Source: CAD feature listing. Evaluate the final solid. Frame: model axes, mm. Face numbers are marked on the shaded views. Give positions to 0.01 mm unless a question says otherwise; leave off trailing zeros. Loops run counter-clockwise (first coordinate to the right, second up) from the corner with the lowest first, then second, coordinate; pieces in that order, holes last. Notation, with made-up numbers: M 24,-25 L 73,-25 A20 cw 73,-13 Z; hole C 84.5,10 d2. An arc over 180 degrees is marked long. Put each result on its own line as item: value.
from build123d import *

# Parameters (mm, degrees)
SKETCH1_R           = 95
SKETCH1_R_2         = 67.5
BOSS_EXTRUDE1_DEPTH = 25
CUT_EXTRUDE1_START  = -10
SKETCH2_R           = 95
SKETCH2_R_2         = 90
CUT_EXTRUDE1_DEPTH  = 10
SKETCH3_R           = 5.75
CUT_EXTRUDE2_DEPTH  = 17.5
CHAMFER1_SIZE       = 2


with BuildPart() as part:
    # Sketch1 → Boss-Extrude1 (new body)
    with BuildSketch(Plane(origin=(0, 0, 0), x_dir=(0, 0, -1), z_dir=(1, 0, 0))):
        Circle(SKETCH1_R)
        Circle(SKETCH1_R_2, mode=Mode.SUBTRACT)
    extrude(amount=BOSS_EXTRUDE1_DEPTH)

    # Sketch2 → Cut-Extrude1 (cut)
    with BuildSketch(Plane(origin=(25, 0, 0), x_dir=(0, 0, -1), z_dir=(1, 0, 0)).offset(CUT_EXTRUDE1_START)):
        Circle(SKETCH2_R)
        Circle(SKETCH2_R_2, mode=Mode.SUBTRACT)
    extrude(amount=CUT_EXTRUDE1_DEPTH, mode=Mode.SUBTRACT)

    # Sketch3 → Cut-Extrude2 (cut)
    with BuildSketch(Plane.ZY):
        with Locations((40.25, -69.715045005)):
            Circle(SKETCH3_R)
        with Locations((80.5, 0)):
            Circle(SKETCH3_R)
        with Locations((-40.25, -69.715045005)):
            Circle(SKETCH3_R)
        with Locations((-80.5, 0)):
            Circle(SKETCH3_R)
        with Locations((-40.25, 69.715045005)):
            Circle(SKETCH3_R)
        with Locations((40.25, 69.715045005)):
            Circle(SKETCH3_R)
    extrude(amount=-CUT_EXTRUDE2_DEPTH, mode=Mode.SUBTRACT)

    # Chamfer1
    chamfer1_edges = [part.edges().sort_by_distance(p)[0] for p in [
        (25, 0, 90),
        (0, 0, 67.5),
    ]]
    chamfer(chamfer1_edges, length=CHAMFER1_SIZE)


solid = part.part
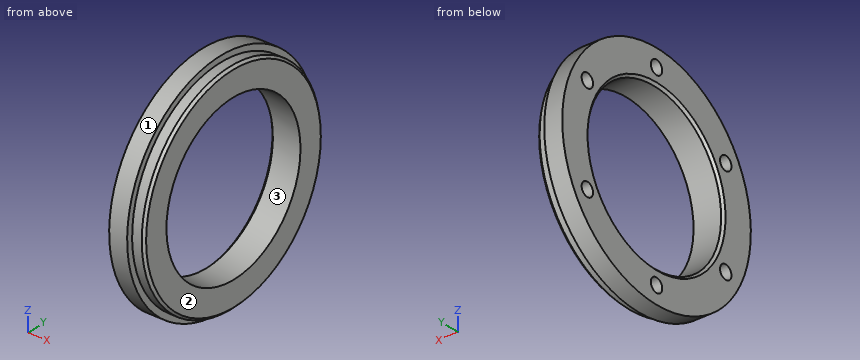
1. Section query A-A (y = 0). Output: boundary loops of the cut face in (x, z), plus the area to 4 significant figures.
Found:
outline: M 0,-95 L 15,-95 L 15,-90 L 23,-90 L 25,-88 L 25,-67.5 L 2,-67.5 L 0,-69.5 L 0,-74.75 L 17.5,-74.75 L 17.5,-86.25 L 0,-86.25 Z; M 0,69.5 L 2,67.5 L 25,67.5 L 25,88 L 23,90 L 15,90 L 15,95 L 0,95 L 0,86.25 L 17.5,86.25 L 17.5,74.75 L 0,74.75 Z
area: 864.5 mm^2
2. Contact query for flat-ended pins moving along their axis: P1, Ø1, axis at x = 5.5, y = 28, coming from the +Z side; P2, Ø1, axis at x = 12, y = -21, coming from the -Z side; P3, Ø4, axis at x = 16.5, y = 19, coming from the +Z side. Output: stop coordinate, or through.
Found:
P1: z = 90.93
P2: z = -92.76
P3: z = 93.34
3. Draft query along Z for the marked faces 1, 2 and 3. Return one class per face: pulls with the +Z half, pulls with the -Z half, needs draft (parallel to the pull), parting line crosses it, or undercut.
Found:
face 1: parting line crosses it
face 2: needs draft
face 3: undercut
4. Material intervals for line 1 (Y direction, x = 7.5, z = 40.25); line 2 (Z direction, x = 11.25, y = 72); line 3 (Z direction, x = 17, y = -72), sorted ascending. Write a range as from..to.
Found:
line 1: -86.05..-75.47, -63.97..-54.19, 54.19..63.97, 75.47..86.05
line 2: -61.98..-45.53, -34.97..34.97, 45.53..61.98
line 3: -54..-45.53, -34.97..34.97, 45.53..54
